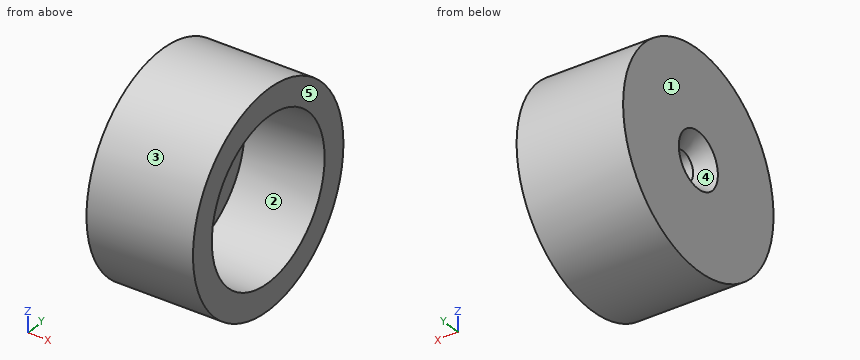
from build123d import *

# Parameters (mm, degrees)
COUNTERSUNK_CENTRE_HOLE_D                     = 6.858
COUNTERSUNK_CENTRE_HOLE_DEPTH                 = 19.05
COUNTERSUNK_CENTRE_HOLE_CSINK_D               = 13.208
COUNTERSUNK_CENTRE_HOLE_CSINK_ANGLE           = 82
COUNTERSUNK_CENTRE_HOLE_TIP                   = 2.060351063
COUNTERSUNK_CENTRE_HOLE_ON_FACE_2_D           = 6.858
COUNTERSUNK_CENTRE_HOLE_ON_FACE_2_DEPTH       = 19.05
COUNTERSUNK_CENTRE_HOLE_ON_FACE_2_CSINK_D     = 13.208
COUNTERSUNK_CENTRE_HOLE_ON_FACE_2_CSINK_ANGLE = 82
COUNTERSUNK_CENTRE_HOLE_ON_FACE_2_TIP         = 2.060351063


with BuildPart() as part:
    # Cup Profile Sketch → Cup Body Revolve (revolve)
    with BuildSketch(Plane.XY):
        Polygon((-19.05, 0), (-25.4, 0), (-25.4, 25.4), (0, 25.4), (0, 19.05), (-19.05, 19.05), align=None)
    revolve(axis=Axis((-19.05, 0, 0), (-1, 0, 0)))

    # Countersunk Centre Hole
    with Locations(Plane(origin=(-25.4, 0, 0), x_dir=(0, -1, 0), z_dir=(-1, 0, 0))):
        with Locations((0, 0)):
            CounterSinkHole(COUNTERSUNK_CENTRE_HOLE_D / 2, COUNTERSUNK_CENTRE_HOLE_CSINK_D / 2, depth=COUNTERSUNK_CENTRE_HOLE_DEPTH, counter_sink_angle=COUNTERSUNK_CENTRE_HOLE_CSINK_ANGLE)
            with Locations((0, 0, -(COUNTERSUNK_CENTRE_HOLE_DEPTH + COUNTERSUNK_CENTRE_HOLE_TIP / 2))):  # 118° drill point
                Cone(0, COUNTERSUNK_CENTRE_HOLE_D / 2, COUNTERSUNK_CENTRE_HOLE_TIP, mode=Mode.SUBTRACT)

    # Countersunk Centre Hole on face 2
    with Locations(Plane(origin=(0, 0, 0), x_dir=(0, -1, 0), z_dir=(-1, 0, 0))):
        with Locations((0, 0)):
            CounterSinkHole(COUNTERSUNK_CENTRE_HOLE_ON_FACE_2_D / 2, COUNTERSUNK_CENTRE_HOLE_ON_FACE_2_CSINK_D / 2, depth=COUNTERSUNK_CENTRE_HOLE_ON_FACE_2_DEPTH, counter_sink_angle=COUNTERSUNK_CENTRE_HOLE_ON_FACE_2_CSINK_ANGLE)
            with Locations((0, 0, -(COUNTERSUNK_CENTRE_HOLE_ON_FACE_2_DEPTH + COUNTERSUNK_CENTRE_HOLE_ON_FACE_2_TIP / 2))):  # 118° drill point
                Cone(0, COUNTERSUNK_CENTRE_HOLE_ON_FACE_2_D / 2, COUNTERSUNK_CENTRE_HOLE_ON_FACE_2_TIP, mode=Mode.SUBTRACT)


solid = part.part
The model under review builds one solid part; all positions refer to its coordinate system, in mm. Face numbers are marked on the shaded views. A direction names the side the tool comes from. Round coordinates to 2 decimals unless told otherwise and drop trailing zeros. Write each loop counter-clockwise with the first axis right and the second up, starting at its lowest first coordinate (ties: lowest second). Pieces come first, ordered by that corner, then holes. Notation, with made-up numbers: (21.5, 78.25) -> (51.5, 78.25) arc R22 cw to (51.5, 87.25) -> close; hole circle Ø11 at (16, 71.25). An arc over 180 degrees is marked (long way). Answer as a JSON object with one key per item and string values.
1. Clearance check with flat-ended pins moving along their axes: pin 1 (6 mm diameter, centred on x = -11.5, z = -9.5, fed in from -Y); pin 2 (1 mm diameter, centred on x = -21.5, y = -10.5, fed in from -Z); pin 3 (8 mm diameter, centred on x = -9, z = 17.5, fed in from -Y). State where each tip first meets the part, or that it passes through.
Results found:
{"pin 1": "stops at y = -24.55", "pin 2": "stops at z = -23.35", "pin 3": "stops at y = -21.52"}
2. We need section C-C on x = -15. State the section outline as (y, z) points.
Results found:
{"outline": "circle Ø50.8 at (0, 0); hole circle Ø38.1 at (0, 0)"}
3. We need section A-A on z = 0. State the section outline as (x, y) points, and give its area (3 significant figures).
Results found:
{"outline": "(-25.4, -25.4) -> (0, -25.4) -> (0, -19.05) -> (-19.05, -19.05) -> (-19.05, -3.43) -> (-21.75, -3.43) -> (-25.4, -6.6) -> close; (-25.4, 6.6) -> (-21.75, 3.43) -> (-19.05, 3.43) -> (-19.05, 19.05) -> (0, 19.05) -> (0, 25.4) -> (-25.4, 25.4) -> close", "area": "509 mm^2"}
4. The part is to be moulded in two halves that separate along Z. For the marked faces 3, 4 and 5, say which applies: pulls with the +Z half, pulls with the -Z half, needs draft (parallel to the pull), parting line crosses it, or undercut.
Results found:
{"face 3": "parting line crosses it", "face 4": "undercut", "face 5": "needs draft"}
5. Machinability: for the marked faces 1 and 2, which of the approach directions +Z, -Z, +X, -X, +Y, -Y give a long, thin tool a straight path to every point of the face, cutting with its end or side? Answer none if there is none.
Results found:
{"face 1": "+Z, -Z, -X, +Y, -Y", "face 2": "+X"}
6. To check wall thickness, follow line 1 along Z through (x, y) = (-6.75, 0); line 2 along Z through (x, y) = (-20.4, 0). State the ranges of each line that lie inside material, in increasing order.
Results found:
{"line 1": "z = -25.4 to -19.05, 19.05 to 25.4", "line 2": "z = -25.4 to -3.43, 3.43 to 25.4"}
7. We need section D-D on z = -10. State the section outline as (x, y) points.
Results found:
{"outline": "(-25.4, -23.35) -> (0, -23.35) -> (0, -16.21) -> (-19.05, -16.21) -> (-19.05, 16.21) -> (0, 16.21) -> (0, 23.35) -> (-25.4, 23.35) -> close"}
